Design review of the part built by this model. Coordinates are the model's own, in mm. Coordinates: 2 decimals unless noted, no trailing zeros. Loops run counter-clockwise (first coordinate to the right, second up) from the corner with the lowest first, then second, coordinate; pieces in that order, holes last. Notation, with made-up numbers: (-16, 45.25) - (5, 45.25) arc R31 ccw to (5, 71.25) - close; hole circle Ø9 at (74.5, 67.5). An arc over 180 degrees is marked (long way). Answer in a Markdown table with one row per item. Add a question column.
(1) To check wall thickness, follow L1, parallel to Z at x = 5.5, y = -59; L2, parallel to Z at x = 6.5, y = 86; L3, parallel to Y at x = 0.75, z = 25. State the ranges of each line that lie inside material, in increasing order. Write a range as [from, to].
(2) Clearance check with flat-ended pins moving along their axes: pin 1 (3 mm diameter, centred on x = 3.5, z = 19, fed in from +Y); pin 2 (5 mm diameter, centred on x = 3.5, y = 52, fed in from -Z); pin 3 (1.5 mm diameter, centred on x = 4, y = 52, fed in from -Z). State where each tip first meets the part, or that it passes through.
(3) We need section A-A, the plane x = 3.5. Write out the cut boundary in (y, z).
(4) We need section B-B, the plane z = -35. Write out the cut boundary in (x, y), plus the area to 3 significant figures.
(5) We need section C-C, the plane y = 61. Write out the cut boundary in (x, z), plus the area to 3 significant figures.
from build123d import *

# Parameters (mm, degrees)
BOSS_EXTRUDE1_DEPTH = 10


with BuildPart() as part:
    # Sketch1 → Boss-Extrude1 (new body)
    with BuildSketch(Plane(origin=(0, 0, 0), x_dir=(0, 0, -1), z_dir=(1, 0, 0))):
        Polygon((40, -80), (-20, 100), (-40, 100), (-40, -80), (-20, -100), (40, -100), align=None)
    extrude(amount=BOSS_EXTRUDE1_DEPTH)


solid = part.part
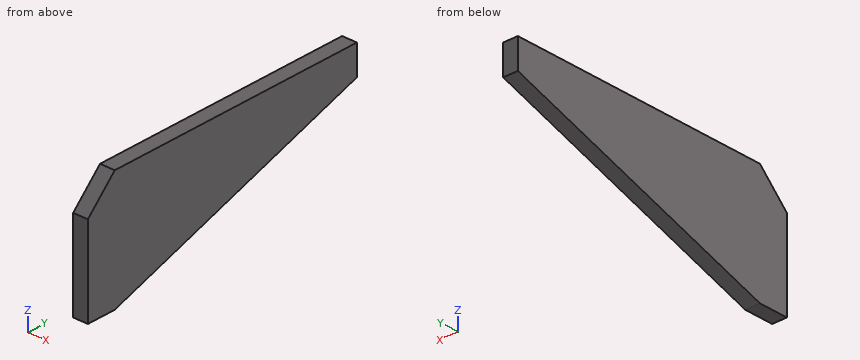
Responses:
| question | item | result |
|---|---|---|
| 1 | L1 | z = [-33, 40] |
| 1 | L2 | z = [15.33, 40] |
| 1 | L3 | y = [-95, 100] |
| 2 | pin 1 | stops at y = 100 |
| 2 | pin 2 | stops at z = 3.17 |
| 2 | pin 3 | stops at z = 3.75 |
| 3 | outline | (-100, -40) - (-80, -40) - (100, 20) - (100, 40) - (-80, 40) - (-100, 20) - close |
| 4 | outline | (0, -100) - (10, -100) - (10, -65) - (0, -65) - close |
| 4 | area | 350 mm2 |
| 5 | outline | (0, 7) - (10, 7) - (10, 40) - (0, 40) - close |
| 5 | area | 330 mm2 |
